Design review of the part built by this model. Coordinates are the model's own, in mm. Face numbers are marked on the shaded views. A direction names the side the tool comes from. Coordinates: 2 decimals unless noted, no trailing zeros. Write each loop counter-clockwise with the first axis right and the second up, starting at its lowest first coordinate (ties: lowest second). Pieces come first, ordered by that corner, then holes. Notation, with made-up numbers: (-35.75, 33) - (-30.75, 33) arc R11 ccw to (-30.75, 49) - close; hole circle Ø4 at (-34, 30). An arc over 180 degrees is marked (long way). Answer as a JSON object with one key per item and string values.
```python
from build123d import *

# Parameters (mm, degrees)
SKETCH_1_W          = 2.75
SKETCH_1_H          = 3
SKETCH_2_R          = 1.5
EXTRUDE_1_DEPTH     = 8
CUT_EXTRUDE_1_DEPTH = 1.5
CHAMFER_1_SIZE      = 0.275


with BuildPart() as part:
    # 草图1 → 旋转1 (revolve)
    with BuildSketch(Plane(origin=(0, 0, 0), x_dir=(1, 0, 0), z_dir=(0, 1, 0))):
        with Locations((1.375, -1.5)):
            Rectangle(SKETCH_1_W, SKETCH_1_H)
    revolve(axis=Axis((0, 0, 0), (0, 0, 1)))

    # 草图2 → 凸台-拉伸1 (add)
    with BuildSketch(Plane(origin=(0, 0, 0), x_dir=(-1, 0, 0), z_dir=(0, 0, -1))):
        Circle(SKETCH_2_R)
    extrude(amount=EXTRUDE_1_DEPTH)

    # 草图3 → 切除-拉伸1 (cut)
    with BuildSketch(Plane.XY.offset(3)):
        Polygon((1.25, -0.721687836), (1.25, 0.721687836), (0, 1.443375673), (-1.25, 0.721687836), (-1.25, -0.721687836), (0, -1.443375673), align=None)
    extrude(amount=-CUT_EXTRUDE_1_DEPTH, mode=Mode.SUBTRACT)

    # 草图4 → 切除-旋转1 (revolve, cut)
    with BuildSketch(Plane.XZ):
        Polygon((1.25, 1.5), (0, 1.5), (0, 0.778312164), align=None)
    revolve(axis=Axis((0, 0, 1.5), (0, 0, -1)), mode=Mode.SUBTRACT)

    # 倒角1
    chamfer_1_edges = [part.edges().sort_by_distance(p)[0] for p in [
        (-2.75, 0, 3),
        (1.5, 0, -8),
    ]]
    chamfer(chamfer_1_edges, length=CHAMFER_1_SIZE)


solid = part.part
```
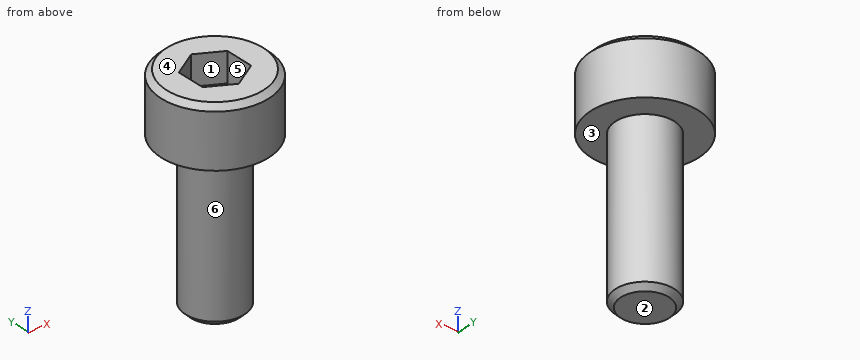
(1) Take a section at A-A, the plane z = 1.75. Write out the cut boundary in (x, y).
Solved:
{"outline": "circle Ø5.5 at (0, 0); hole (-1.25, -0.72) - (0, -1.44) - (1.25, -0.72) - (1.25, 0.72) - (0, 1.44) - (-1.25, 0.72) - close"}
(2) Take a section at B-B, the plane z = -7.5. Write out the cut boundary in (x, y).
Solved:
{"outline": "circle Ø3 at (0, 0)"}
(3) For pin 1 (2 mm diameter, centred on y = -1.5, z = -3, fed in from +X); pin 2 (1 mm diameter, centred on x = 0, z = -2.5, fed in from +Y); pin 3 (1 mm diameter, centred on x = 0.5, z = -3, fed in from -Y), all flat-tipped, find the tip position at first contact; note any pin that passes through.
Solved:
{"pin 1": "stops at x = 1.41", "pin 2": "stops at y = 1.5", "pin 3": "stops at y = -1.5"}
(4) To check wall thickness, follow line 1 (Z direction, x = 0.55, y = -2.3); line 2 (Y direction, x = 0.1, z = -6.5); line 3 (X direction, y = -1.35, z = 2.25). State the ranges of each line that lie inside material, in increasing order. Write a range as from..to.
Solved:
{"line 1": "z = 0..3", "line 2": "y = -1.5..1.5", "line 3": "x = -2.4..-0.16, 0.16..2.4"}
(5) The part is to be moulded in two halves that separate along Y. For the marked faces 4, 5 and 6, say which applies: pulls with the +Y half, pulls with the -Y half, needs draft (parallel to the pull), parting line crosses it, or undercut.
Solved:
{"face 4": "needs draft", "face 5": "undercut", "face 6": "parting line crosses it"}
(6) Tool access review of the marked faces 1, 2 and 3: name each direction out of +Z, -Z, +X, -X, +Y, -Y from which nothing blocks a thin tool from reaching the whole face with its end or side.
Solved:
{"face 1": "+Z", "face 2": "-Z, +X, -X, +Y, -Y", "face 3": "-Z"}
(7) Take a section at C-C, the plane z = 0.5. Write out the cut boundary in (x, y).
Solved:
{"outline": "circle Ø5.5 at (0, 0)"}
